from build123d import *

# Parameters (mm, degrees)
SKETCH_2_W             = 520
SKETCH_2_H             = 65
EXTRUDE_1_DEPTH        = 12
HOLE_WIZARD_7_0_7_1_D  = 7
CHAMFER_1_SIZE         = 3
HOLE_WIZARD_9_0_9_2_D  = 9
HOLE_WIZARD_9_0_9_1_D  = 7
PATTERN_LINEAR_1_COUNT = 2
PATTERN_LINEAR_1_PITCH = 115
HOLE_WIZARD_9_0_9_3_D  = 9
HOLE_WIZARD_M5_1_D     = 4.2
HOLE_WIZARD_M5_1_DEPTH = 12.4
HOLE_WIZARD_M5_1_TIP   = 1.2618073
HOLE_WIZARD_M5_2_D     = 4.2
HOLE_WIZARD_M5_2_DEPTH = 12.4
HOLE_WIZARD_M5_2_TIP   = 1.2618073


with BuildPart() as part:
    # 草图2 → 凸台-拉伸1 (new body)
    with BuildSketch(Plane(origin=(0, 0, 0), x_dir=(1, 0, 0), z_dir=(0, 1, 0))):
        Rectangle(SKETCH_2_W, SKETCH_2_H)
    extrude(amount=EXTRUDE_1_DEPTH)

    # Ø7.0 (7) 直径孔1 (through all)
    with Locations(Plane.XZ):
        with Locations((240, -20), (200, -20), (200, 20), (240, 20)):
            Hole(HOLE_WIZARD_7_0_7_1_D / 2)

    # 倒角1
    chamfer_1_edges = [part.edges().sort_by_distance(p)[0] for p in [
        (260, 6, 32.5),
        (-260, 6, 32.5),
        (-260, 6, -32.5),
        (260, 6, -32.5),
    ]]
    chamfer(chamfer_1_edges, length=CHAMFER_1_SIZE)

    # Ø9.0 (9) 直径孔2 (through all)
    with Locations(Plane(origin=(0, 12, 0), x_dir=(1, 0, 0), z_dir=(0, 1, 0))):
        with Locations((-160, -22.5), (-160, 22.5)):
            Hole(HOLE_WIZARD_9_0_9_2_D / 2)

    # Ø9.0 (9) 直径孔1 (through all)
    with Locations(Plane(origin=(0, 12, 0), x_dir=(1, 0, 0), z_dir=(0, 1, 0))):
        with Locations((-235, -17.5), (-235, 17.5), (-200, -17.5), (-200, 17.5)):
            hole_wizard_9_0_9_1 = Hole(HOLE_WIZARD_9_0_9_1_D / 2)

    # 阵列(线性)1: Ø9.0 (9) 直径孔1 ×2
    with Locations(*[(i * PATTERN_LINEAR_1_PITCH, 0, 0) for i in range(1, PATTERN_LINEAR_1_COUNT)]):
        add(hole_wizard_9_0_9_1, mode=Mode.SUBTRACT)

    # Ø9.0 (9) 直径孔3 (through all)
    with Locations(Plane(origin=(0, 12, 0), x_dir=(1, 0, 0), z_dir=(0, 1, 0))):
        with Locations((-45, -22.5), (-45, 22.5)):
            Hole(HOLE_WIZARD_9_0_9_3_D / 2)

    # M5 螺纹孔1
    with Locations(Plane(origin=(0, 0, -32.5), x_dir=(-1, 0, 0), z_dir=(0, 0, -1))):
        with Locations((95, 6), (110, 6)):
            Hole(HOLE_WIZARD_M5_1_D / 2, depth=HOLE_WIZARD_M5_1_DEPTH)
            with Locations((0, 0, -(HOLE_WIZARD_M5_1_DEPTH + HOLE_WIZARD_M5_1_TIP / 2))):  # 118° drill point
                Cone(0, HOLE_WIZARD_M5_1_D / 2, HOLE_WIZARD_M5_1_TIP, mode=Mode.SUBTRACT)

    # M5 螺纹孔2
    with Locations(Plane.XY.offset(32.5)):
        with Locations((-95, 6), (-110, 6)):
            Hole(HOLE_WIZARD_M5_2_D / 2, depth=HOLE_WIZARD_M5_2_DEPTH)
            with Locations((0, 0, -(HOLE_WIZARD_M5_2_DEPTH + HOLE_WIZARD_M5_2_TIP / 2))):  # 118° drill point
                Cone(0, HOLE_WIZARD_M5_2_D / 2, HOLE_WIZARD_M5_2_TIP, mode=Mode.SUBTRACT)


solid = part.part
For this review, take the finished solid that the model builds, in its own axes (mm). Round coordinates to 2 decimals unless told otherwise and drop trailing zeros. Write item = value, one per line. Start each with the question number.
1) To check wall thickness, follow line 1 (Z direction, x = -45, y = 8.25); line 2 (X direction, y = 6, z = -29); line 3 (X direction, y = 3, z = 21.5). State the ranges of each line that lie inside material, in increasing order. Write a range as from..to.
2) Insertion check: pin 1 (5.5 mm diameter, centred on x = -160, z = 22.5, fed in from -Y); pin 2 (3.5 mm diameter, centred on x = -95, y = 6, fed in from -Z); pin 3 (2.5 mm diameter, centred on x = -110, y = 6, fed in from -Z); pin 4 (2.5 mm diameter, centred on x = -110, y = 6, fed in from +Z). Each pin has a flat end and moves straight along its axis. Give the tip position at first contact, or say it passes through.
3) The part is to be moulded in two halves that separate along X. For faces 1 (the face through (-164.292, 5.916, -23.852)), 2 (the face through (-260, 6, 0)), 3 (the face through (-4, 12, 0)), 4 (the face through (260, 6, 0)), say which applies: +X half, -X half, draft (parallel to the pull), parting line (faces both ways), or undercut.
Verdict:
q1.line_1 = -32.5..-27, -18..18, 27..32.5
q1.line_2 = -260..-112.1, -107.9..-97.1, -92.9..260
q1.line_3 = -260..-164.39, -155.61..-49.39, -40.61..196.84, 203.16..236.84, 243.16..260
q2.pin_1 = through
q2.pin_2 = -19.89
q2.pin_3 = -19.59
q2.pin_4 = 19.59
q3.face_1 = undercut
q3.face_2 = -X half
q3.face_3 = draft
q3.face_4 = +X half
